from build123d import *

# Parameters (mm, degrees)
SKETCH1_R           = 3
SKETCH1_R_2         = 4
BOSS_EXTRUDE1_DEPTH = 5
SKETCH2_R           = 13
CUT_EXTRUDE1_DEPTH  = 2
SKETCH4_R           = 1.25
BOSS_EXTRUDE2_DEPTH = 2
BOSS_EXTRUDE3_START = 20
SKETCH5_R           = 15
SKETCH5_R_2         = 13
BOSS_EXTRUDE3_DEPTH = 20


with BuildPart() as part:
    # Sketch1 → Boss-Extrude1 (new body)
    with BuildSketch(Plane.XY):
        with BuildLine():
            Line((4.437522393, -8.961495132), (32.27272364, -32.382887973))
            ThreePointArc((32.27272364, -32.382887973), (57.387408796, -48.287527496), (37.423393239, -26.261564368))
            Line((37.423393239, -26.261564368), (9.588191993, -2.840171527))
            ThreePointArc((9.588191993, -2.840171527), (-7.651654506, 6.438336999), (4.437522393, -8.961495132))
        make_face()
        Circle(SKETCH1_R, mode=Mode.SUBTRACT)
        with Locations((45.909927037, -38.630021997)):
            Circle(SKETCH1_R_2, mode=Mode.SUBTRACT)
    extrude(amount=BOSS_EXTRUDE1_DEPTH)

    # Sketch2 → Cut-Extrude1 (cut)
    with BuildSketch(Plane(origin=(0, 0, 0), x_dir=(-1, 0, 0), z_dir=(0, 0, -1))):
        with Locations((-45.909927037, -38.630021997)):
            Circle(SKETCH2_R)
    extrude(amount=-CUT_EXTRUDE1_DEPTH, mode=Mode.SUBTRACT)

    # Sketch4 → Boss-Extrude2 (add)
    with BuildSketch(Plane(origin=(0, 0, 0), x_dir=(-1, 0, 0), z_dir=(0, 0, -1))):
        with Locations((-45.909927037, -25.630021997)):
            Circle(SKETCH4_R)
        with Locations((-57.168257286, -45.130021997)):
            Circle(SKETCH4_R)
        with Locations((-34.651596788, -45.130021997)):
            Circle(SKETCH4_R)
    extrude(amount=-BOSS_EXTRUDE2_DEPTH)

    # Sketch5 → Boss-Extrude3 (add)
    with BuildSketch(Plane(origin=(0, 0, 0), x_dir=(-1, 0, 0), z_dir=(0, 0, -1)).offset(BOSS_EXTRUDE3_START)):
        with Locations((-45.909927037, -38.630021997)):
            Circle(SKETCH5_R)
        with Locations((-45.909927037, -38.630021997)):
            Circle(SKETCH5_R_2, mode=Mode.SUBTRACT)
    extrude(amount=-BOSS_EXTRUDE3_DEPTH)


solid = part.part
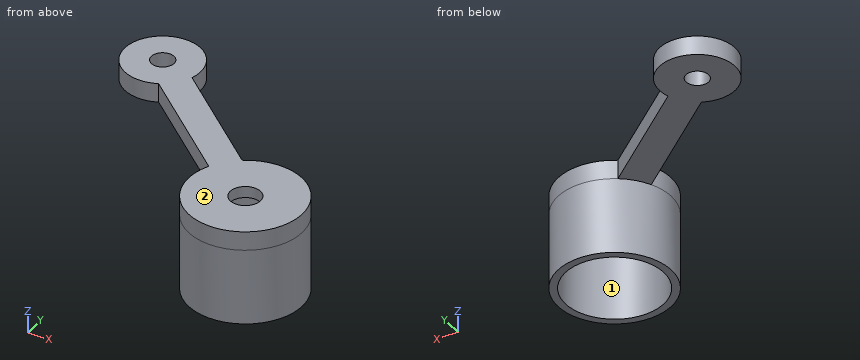
Verification items for the finished model (mm, model axes). Face numbers are marked on the shaded views. Coordinates: 2 decimals unless noted, no trailing zeros. Order: outer loops, then holes, each group sorted by start corner. A loop starts at its lowest first (then second) coordinate and runs counter-clockwise, first axis right, second up. Notation, with made-up numbers: M -31.75,-35.75 L 25.25,-35.75 A25 cw 25.25,-7.75 Z; hole C 25.5,-24.5 d8. An arc over 180 degrees is marked long. Write each question's results on one line, items separated by ' | '.
1) Section check C-C on y = -36.5. Record the cut outline in (x, z).
Solved:
outline: M 31.06,-20 L 33.09,-20 L 33.09,2 L 42.52,2 L 42.52,5 L 31.06,5 Z; M 49.3,2 L 58.73,2 L 58.73,-20 L 60.76,-20 L 60.76,5 L 49.3,5 Z
2) Gauge pin test, flat ends, axial feed: pin 1 Ø12 at (x, y) = (17.5, -20) entering from -Z; pin 2 Ø8 at (y, z) = (-22.5, -9) entering from -X; pin 3 Ø8 at (x, z) = (45.5, -14.5) entering from +Y. Record the tip position at first contact, or that the pin passes through.
Solved:
pin 1: stops at z = 0 | pin 2: stops at x = 37.09 | pin 3: stops at y = -23.63
3) Section check A-A on y = 0. Record the cut outline in (x, z).
Solved:
outline: M -10,0 L -3,0 L -3,5 L -10,5 Z; M 3,0 L 10,0 L 10,5 L 3,5 Z
4) Scan lines: line 1 along Y through (x, z) = (0, 2.75); line 2 along Z through (x, y) = (-3.5, -4); line 3 along Y through (x, z) = (44, -9). Record each from-to range of solid material in increasing order. Write a range as [from, to].
Solved:
line 1: y = [-10, -3], [3, 10] | line 2: z = [0, 5] | line 3: y = [-53.51, -51.49], [-25.77, -23.75]
5) Section check D-D on z = -16.75. Record the cut outline in (x, y), plus the area to 3 significant figures.
Solved:
outline: C 45.91,-38.63 d30; hole C 45.91,-38.63 d26 | area: 176 mm²
6) Release check for a two-part mould opening along X. For the marked faces 1 and 2 record: pulls with the +X half, pulls with the -X half, needs draft (parallel to the pull), parting line crosses it, or undercut.
Solved:
face 1: undercut | face 2: needs draft
